Build history of the part. All positions in model axes, mm. A direction names the side the tool comes from. Round coordinates to 2 decimals unless told otherwise and drop trailing zeros. Write each loop counter-clockwise with the first axis right and the second up, starting at its lowest first coordinate (ties: lowest second). Pieces come first, ordered by that corner, then holes.
1) Pull direction Y, two halves, no side cores. Call faces 4 (the flat face through (0, 138, -16)), 5 (the cylindrical face through (80.12, 51.08, -8.87)), 6 (the cylindrical face through (61.35, 178.99, -73.36)), 7 (the flat face through (49, 200, -59)): +Y half, -Y half, draft (parallel to the pull), parting line (faces both ways), or undercut.
2) Saw through at C-C (z = -75). Write the cut outline in (x, y).
3) Saw through at A-A (x = 15). State how many separate pieces and enclosed holes the cut face has, plus the area to 3 significant figures.
4) Flat gauge pins, fed straight in: pin 1 (12 mm diameter, centred on y = 34.5, z = -36.5, fed in from +X); pin 2 (4 mm diameter, centred on x = 26, z = -93, fed in from -Y); pin 3 (16 mm diameter, centred on x = 23, y = 54.5, fed in from -Z). Where does each tip first touch, or does it go through?
5) Saw through at B-B (y = 15). Write the cut outline in (x, z), plus the area to 3 significant figures.
6) Saw through at D-D (z = -110). Write the cut outline in (x, y).
7) Which spindle directions (+Z, -Z, +X, -X, +Y, -Y) get a long thin tool onto all of the face, cutting with end or side? Do faces 1 (the flat face through (100, 138, -16)), 2 (the flat face through (23, 182, -75)), 3 (the cylindrical face through (84.47, 179.15, -21.01)). Say none if no direction does.
8) Wall check: probe 1 along Y at (x, z) = (15, -9); probe 2 along X at (y, z) = (189, -100); probe 3 along Y at (x, z) = (27.5, -42). Give the ranges that are in metal, low to high.
from build123d import *

# Parameters (mm, degrees)
BOSS_EXTRUDE1_DEPTH = 100
FILLET1_R           = 10
RIB3_REACH          = 240.537
SKETCH2_WALL_W      = 687.708067886
SKETCH2_WALL_H      = 17
FILLET2_R           = 10
SKETCH3_R           = 6
SKETCH3_R_2         = 5
CUT_EXTRUDE2_DEPTH  = 254.771550809
SKETCH7_R           = 6
SKETCH7_R_2         = 5
CUT_EXTRUDE3_DEPTH  = 254.771550809


with BuildPart() as part:
    # Sketch1 → Boss-Extrude1 (new body)
    with BuildSketch(Plane(origin=(0, 0, 0), x_dir=(0, 0, -1), z_dir=(1, 0, 0))):
        Polygon((0, 0), (0, 200), (120, 200), (120, 182), (18, 182), (18, 0), align=None)
    extrude(amount=BOSS_EXTRUDE1_DEPTH)

    # Fillet1
    fillet1_edges = [part.edges().sort_by_distance(p)[0] for p in [
        (50, 182, -18),
    ]]
    fillet(fillet1_edges, radius=FILLET1_R)

    # Sketch2 wall → Rib3 (add, up to next)
    with BuildSketch(Plane(origin=(50, 91, -69), x_dir=(0, -0.87234249996, 0.48889524723), z_dir=(0, -0.48889524723, -0.87234249996)), mode=Mode.PRIVATE) as rib3_sk1:
        Rectangle(SKETCH2_WALL_W, SKETCH2_WALL_H)
    rib3_tool1 = extrude(rib3_sk1.sketch, amount=-RIB3_REACH, mode=Mode.PRIVATE) - part.part
    add(rib3_tool1.solids().sort_by_distance((50, 91, -69))[0])

    # Fillet2
    fillet2_edges = [part.edges().sort_by_distance(p)[0] for p in [
        (41.5, 179.071067812, -20.928932188),
        (58.5, 179.071067812, -20.928932188),
        (41.5, 86, -18),
        (41.5, 182, -74),
        (58.5, 182, -74),
        (58.5, 86, -18),
    ]]
    fillet(fillet2_edges, radius=FILLET2_R)

    # Sketch3 → Cut-Extrude2 (cut, through all)
    with BuildSketch(Plane.XY):
        with Locations((15, 15)):
            Circle(SKETCH3_R)
        with Locations((15, 50)):
            Circle(SKETCH3_R_2)
        with Locations((15, 85)):
            Circle(SKETCH3_R)
        with Locations(Location((85, 15, 0), (0, 0, 270))):
            Circle(SKETCH3_R)
        with Locations(Location((85, 50, 0), (0, 0, 270))):
            Circle(SKETCH3_R_2)
        with Locations(Location((85, 85, 0), (0, 0, 270))):
            Circle(SKETCH3_R)
    extrude(amount=-CUT_EXTRUDE2_DEPTH, mode=Mode.SUBTRACT)

    # Sketch7 → Cut-Extrude3 (cut, through all)
    with BuildSketch(Plane(origin=(0, 200, 0), x_dir=(1, 0, 0), z_dir=(0, 1, 0))):
        with Locations(Location((15, 100, 0), (0, 0, 270))):
            Circle(SKETCH7_R)
        with Locations(Location((15, 75, 0), (0, 0, 270))):
            Circle(SKETCH7_R_2)
        with Locations(Location((15, 50, 0), (0, 0, 270))):
            Circle(SKETCH7_R)
        with Locations(Location((85, 50, 0), (0, 0, 270))):
            Circle(SKETCH7_R)
        with Locations(Location((85, 75, 0), (0, 0, 270))):
            Circle(SKETCH7_R_2)
        with Locations(Location((85, 100, 0), (0, 0, 270))):
            Circle(SKETCH7_R)
    extrude(amount=-CUT_EXTRUDE3_DEPTH, mode=Mode.SUBTRACT)


solid = part.part
Evaluation:
1. face 4: draft
1. face 5: undercut
1. face 6: -Y half
1. face 7: +Y half
2. outline: (0, 182) - (10, 182) - (10, 200) - (0, 200) - close; (20, 182) - (31.5, 182) arc R10 cw to (41.5, 172) - (41.5, 101.71) - (58.5, 101.71) - (58.5, 172) arc R10 cw to (68.5, 182) - (80, 182) - (80, 200) - (20, 200) - close; (90, 182) - (100, 182) - (100, 200) - (90, 200) - close
3. separate pieces: 7
3. enclosed holes: 0
3. area: 4,230 mm2
4. pin 1: stops at x = 58.5
4. pin 2: stops at y = 182
4. pin 3: stops at z = -18
5. outline: (0, -18) - (9, -18) - (9, 0) - (0, 0) - close; (21, -18) - (31.5, -18) arc R10 cw to (41.37, -26.41) - (58.63, -26.41) arc R10 cw to (68.5, -18) - (79, -18) - (79, 0) - (21, 0) - close; (91, -18) - (100, -18) - (100, 0) - (91, 0) - close
5. area: 1,550 mm2
6. outline: (0, 182) - (31.5, 182) arc R10 cw to (41.5, 172) - (41.5, 164.16) - (58.5, 164.16) - (58.5, 172) arc R10 cw to (68.5, 182) - (100, 182) - (100, 200) - (0, 200) - close
7. face 1: +Z, -Z, +X, +Y, -Y
7. face 2: -Z, -X, -Y
7. face 3: -Z, +X, -Y
8. probe 1: y = 0 to 9, 21 to 45, 55 to 79, 91 to 200
8. probe 2: x = 0 to 9, 21 to 79, 91 to 100
8. probe 3: y = 182 to 200
